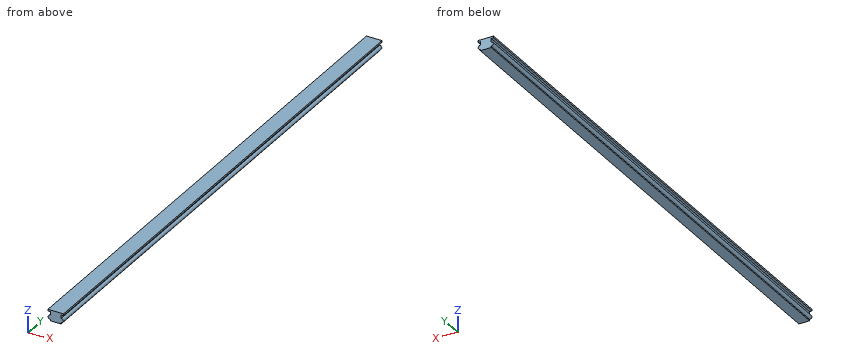
from build123d import *

# Parameters (mm, degrees)
EXTRUDE_1_DEPTH = 1252


with BuildPart() as part:
    # 草图1 → 凸台-拉伸1 (new body)
    with BuildSketch(Plane(origin=(0, 0, 0), x_dir=(1, 0, 0), z_dir=(0, 1, 0))):
        with BuildLine():
            Line((-12.5, 5), (-12.5, 8))
            Line((-12.5, 8), (12.5, 8))
            Line((12.5, 8), (12.5, 5))
            ThreePointArc((12.5, 5), (17.5, 0), (12.5, -5))
            Line((12.5, -5), (12.5, -13))
            Line((12.5, -13), (18, -13))
            Line((18, -13), (18, -17))
            Line((18, -17), (-18, -17))
            Line((-18, -17), (-18, -13))
            Line((-18, -13), (-12.5, -13))
            Line((-12.5, -13), (-12.5, -5))
            ThreePointArc((-12.5, -5), (-17.5, 0), (-12.5, 5))
        make_face()
    extrude(amount=EXTRUDE_1_DEPTH)


solid = part.part
The listing builds one solid part. Answer for the finished solid, in the listing's coordinates (mm). Round coordinates to 2 decimals unless told otherwise and drop trailing zeros. Write each loop counter-clockwise with the first axis right and the second up, starting at its lowest first coordinate (ties: lowest second). Pieces come first, ordered by that corner, then holes. Notation, with made-up numbers: M -31.5,9.25 L -4.5,9.25 A13 ccw -4.5,32.25 Z; hole C 8,69.25 d7. An arc over 180 degrees is marked long. Write each question's results on one line, items separated by ' | '. Start each with the question number.
(1) The part is cut by section A-A, the plane y = 998. Write down the section's boundary in (x, z), and give its area (3 significant figures).
(2) Find the intervals of material crossed by line 1 (Z direction, x = 13.5, y = 592); line 2 (Z direction, x = -14, y = 522); line 3 (X direction, y = 787, z = 0.75), in increasing order.
(3) The part is cut by section B-B, the plane z = 0. Write down the section's boundary in (x, y), and give its area (3 significant figures).
(4) Each of these flat-tipped pins is pushed along its axis until it touches: P1, Ø3, axis at x = 15.5, y = 740, coming from the -Z side; P2, Ø8, axis at x = -13.5, z = -5, coming from the -Y side; P3, Ø4, axis at y = 660, z = 9.5, coming from the +X side; P4, Ø1.6, axis at x = -16, y = 344, coming from the -Z side. Where does it stop, or does it pass through?
Worked answers:
1) outline: M -18,13 L -12.5,13 L -12.5,5 A5 ccw -12.5,-5 L -12.5,-8 L 12.5,-8 L 12.5,-5 A5 ccw 12.5,5 L 12.5,13 L 18,13 L 18,17 L -18,17 Z | area: 748 mm²
2) line 1: z = -4.9 to 4.9, 13 to 17 | line 2: z = -4.77 to 4.77, 13 to 17 | line 3: x = -17.44 to 17.44
3) outline: M -17.5,0 L 17.5,0 L 17.5,1252 L -17.5,1252 Z | area: 43,800 mm²
4) P1: stops at z = -4.77 | P2: stops at y = 0 | P3: stops at x = 12.5 | P4: stops at z = -4.21
